Verification items for this drawing (mm, ordinates from the low corner). A direction names the side the tool comes from. Give positions to 0.01 mm unless a question says otherwise; leave off trailing zeros. Loops run counter-clockwise (first coordinate to the right, second up) from the corner with the lowest first, then second, coordinate; pieces in that order, holes last. Notation, with made-up numbers: M 77,38 L 128,38 A9 cw 128,53 Z; hole C 7.25,58.25 d9. An arc over 180 degrees is marked long. Write each question's results on one line, items separated by ' | '. Start each with the question number.
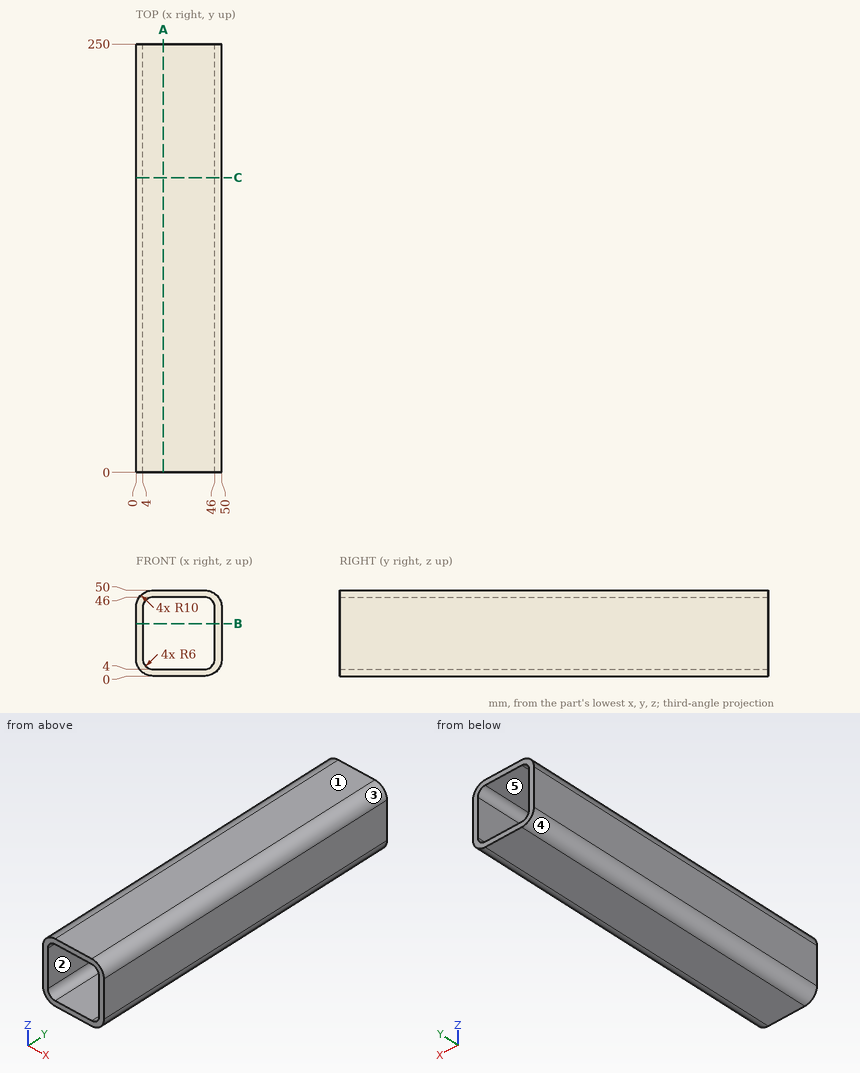
1. Section check A-A, the plane x = 16. Record the boundary of the cut face in (y, z), plus the area to 3 significant figures.
2. Set-up check for the marked faces 4 and 5: record each of +Z, -Z, +X, -X, +Y, -Y from which the full face is reachable in a straight line by a thin tool's end or side.
3. Section check B-B, the plane z = 30.5. Record the boundary of the cut face in (x, y), plus the area to 3 significant figures.
4. Section check C-C, the plane y = 172. Record the boundary of the cut face in (x, z), plus the area to 3 significant figures.
5. Thickness scan on probe 1 along X at (y, z) = (198, 17); probe 2 along X at (y, z) = (67.5, 7). Record the ranges inside material, lowest first.
6. Release check for a two-part mould opening along X. For the marked faces 1, 2 and 3 record: released by +X, released by -X, zero draft, split by the parting line, or undercut.
7. Depth check by flat-ended pin: pin 1 Ø1 at (y, z) = (73, 42) entering from +X; pin 2 Ø2 at (x, z) = (22.5, 5.5) entering from +Y. Enter the tip coordinate at first touch or a pass-through.
Filled sheet:
1) outline: M 0,0 L 250,0 L 250,4 L 0,4 Z; M 0,46 L 250,46 L 250,50 L 0,50 Z | area: 2,000 mm2
2) face 4: -Z, -X, +Y, -Y | face 5: +Y, -Y
3) outline: M 0,0 L 4,0 L 4,250 L 0,250 Z; M 46,0 L 50,0 L 50,250 L 46,250 Z | area: 2,000 mm2
4) outline: M 0,10 A10 ccw 10,0 L 40,0 A10 ccw 50,10 L 50,40 A10 ccw 40,50 L 10,50 A10 ccw 0,40 Z; hole M 4,10 A6 ccw 10,4 L 40,4 A6 ccw 46,10 L 46,40 A6 ccw 40,46 L 10,46 A6 ccw 4,40 Z | area: 681 mm2
5) probe 1: 0 to 4, 46 to 50 | probe 2: 0.46 to 4.8, 45.2 to 49.54
6) face 1: zero draft | face 2: undercut | face 3: released by +X
7) pin 1: x = 49.89 | pin 2: through
